Here's how the part is built. I have some questions about the finished solid (model axes, mm). Round coordinates to 2 decimals unless told otherwise and drop trailing zeros. Loops run counter-clockwise (first coordinate to the right, second up) from the corner with the lowest first, then second, coordinate; pieces in that order, holes last. Notation, with made-up numbers: (9.5, 17) - (35.5, 17) arc R28 cw to (35.5, 41) - close; hole circle Ø2 at (-37.75, 61). An arc over 180 degrees is marked (long way). Answer as a JSON object with one key per item and string values. Group by question number.
1) If I drill on line 1 along Z through (x, y) = (156, -13.5); line 2 along Z through (x, y) = (226, -28); line 3 along X through (y, z) = (-14, 1528), over which ranges is the centre line in solid material (lowest first)? Write a range as [from, to].
2) I want a section at A-A, the plane x = 136.5. Give the number of separate pieces and of enclosed holes in the cut face, then the cut area to 3 significant figures.
3) I want a section at C-C, the plane y = -19. Please give me the cut outline in (x, z), then the cut area to 3 significant figures.
4) I want a section at B-B, the plane z = 458. Please give me the cut outline in (x, y), then the cut area to 3 significant figures.
5) Will these pins go through, and if not, where does the flat tip stop? P1, Ø11.5, axis at y = -9.5, z = 21.5, coming from the +X side; P2, Ø1.1, axis at y = -29, z = 1297, coming from the -X side; P3, Ø3, axis at y = -28.5, z = 89, coming from the -X side.
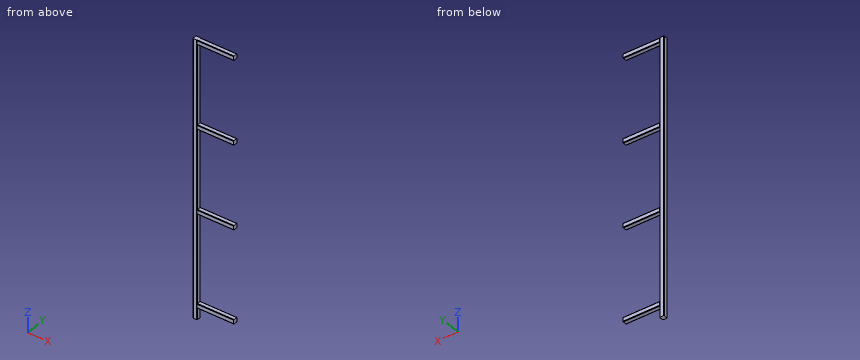
from build123d import *

# Parameters (mm, degrees)
BOSS_EXTRUDE1_DEPTH = 1880
BOSS_EXTRUDE2_DEPTH = 250


with BuildPart() as part:
    # Sketch1 → Boss-Extrude1 (new body)
    with BuildSketch(Plane.XY):
        with BuildLine():
            Line((3.5, 0), (26.5, 0))
            ThreePointArc((26.5, 0), (28.974873734, -1.025126266), (30, -3.5))
            Line((30, -3.5), (30, -26.5))
            ThreePointArc((30, -26.5), (28.974873734, -28.974873734), (26.5, -30))
            Line((26.5, -30), (3.5, -30))
            ThreePointArc((3.5, -30), (1.025126266, -28.974873734), (0, -26.5))
            Line((0, -26.5), (0, -3.5))
            ThreePointArc((0, -3.5), (1.025126266, -1.025126266), (3.5, 0))
        make_face()
    extrude(amount=BOSS_EXTRUDE1_DEPTH)

    # Sketch2 → Boss-Extrude2 (add)
    with BuildSketch(Plane(origin=(30, 0, 0), x_dir=(0, 0, -1), z_dir=(1, 0, 0))):
        with BuildLine():
            Line((-1876.5, 0), (-1853.5, 0))
            ThreePointArc((-1853.5, 0), (-1851.025126266, -1.025126266), (-1850, -3.5))
            Line((-1850, -3.5), (-1850, -26.5))
            ThreePointArc((-1850, -26.5), (-1851.025126266, -28.974873734), (-1853.5, -30))
            Line((-1853.5, -30), (-1876.5, -30))
            ThreePointArc((-1876.5, -30), (-1878.974873734, -28.974873734), (-1880, -26.5))
            Line((-1880, -26.5), (-1880, -3.5))
            ThreePointArc((-1880, -3.5), (-1878.974873734, -1.025126266), (-1876.5, 0))
        make_face()
        with BuildLine():
            Line((-104.561536833, 0), (-81.561536833, 0))
            ThreePointArc((-81.561536833, 0), (-79.086663099, -1.025126266), (-78.061536833, -3.5))
            Line((-78.061536833, -3.5), (-78.061536833, -26.5))
            ThreePointArc((-78.061536833, -26.5), (-79.086663099, -28.974873734), (-81.561536833, -30))
            Line((-81.561536833, -30), (-104.561536833, -30))
            ThreePointArc((-104.561536833, -30), (-107.036410567, -28.974873734), (-108.061536833, -26.5))
            Line((-108.061536833, -26.5), (-108.061536833, -3.5))
            ThreePointArc((-108.061536833, -3.5), (-107.036410567, -1.025126266), (-104.561536833, 0))
        make_face()
        with BuildLine():
            Line((-1306.742108749, 0), (-1283.742108749, 0))
            ThreePointArc((-1283.742108749, 0), (-1281.267235014, -1.025126266), (-1280.242108749, -3.5))
            Line((-1280.242108749, -3.5), (-1280.242108749, -26.5))
            ThreePointArc((-1280.242108749, -26.5), (-1281.267235014, -28.974873734), (-1283.742108749, -30))
            Line((-1283.742108749, -30), (-1306.742108749, -30))
            ThreePointArc((-1306.742108749, -30), (-1309.216982483, -28.974873734), (-1310.242108749, -26.5))
            Line((-1310.242108749, -26.5), (-1310.242108749, -3.5))
            ThreePointArc((-1310.242108749, -3.5), (-1309.216982483, -1.025126266), (-1306.742108749, 0))
        make_face()
        with BuildLine():
            Line((-736.86903894, 0), (-713.86903894, 0))
            ThreePointArc((-713.86903894, 0), (-711.394165206, -1.025126266), (-710.36903894, -3.5))
            Line((-710.36903894, -3.5), (-710.36903894, -26.5))
            ThreePointArc((-710.36903894, -26.5), (-711.394165206, -28.974873734), (-713.86903894, -30))
            Line((-713.86903894, -30), (-736.86903894, -30))
            ThreePointArc((-736.86903894, -30), (-739.343912674, -28.974873734), (-740.36903894, -26.5))
            Line((-740.36903894, -26.5), (-740.36903894, -3.5))
            ThreePointArc((-740.36903894, -3.5), (-739.343912674, -1.025126266), (-736.86903894, 0))
        make_face()
    extrude(amount=BOSS_EXTRUDE2_DEPTH)


solid = part.part
Outcome:
{
 "1": {"line 1": "[78.06, 108.06], [710.37, 740.37], [1280.24, 1310.24], [1850, 1880]", "line 2": "[78.4, 107.72], [710.71, 740.03], [1280.58, 1309.9], [1850.34, 1879.66]", "line 3": "[0, 30]"},
 "2": {"separate pieces": "4", "enclosed holes": "0", "area": "3,560 mm^2"},
 "3": {"outline": "(0, 0) - (30, 0) - (30, 78.06) - (280, 78.06) - (280, 108.06) - (30, 108.06) - (30, 710.37) - (280, 710.37) - (280, 740.37) - (30, 740.37) - (30, 1280.24) - (280, 1280.24) - (280, 1310.24) - (30, 1310.24) - (30, 1850) - (280, 1850) - (280, 1880) - (0, 1880) - close", "area": "86,400 mm^2"},
 "4": {"outline": "(0, -26.5) arc R3.5 ccw to (3.5, -30) - (26.5, -30) arc R3.5 ccw to (30, -26.5) - (30, -3.5) arc R3.5 ccw to (26.5, 0) - (3.5, 0) arc R3.5 ccw to (0, -3.5) - close", "area": "889 mm^2"},
 "5": {"P1": "x = 30", "P2": "x = 0.59", "P3": "x = 0.04"}
}
